```python
from build123d import *

# Parameters (mm, degrees)
SKETCH_1_R      = 23.5
SKETCH_1_R_2    = 8.5
EXTRUDE_1_DEPTH = 15
FILLET_1_R      = 0.8


with BuildPart() as part:
    # 草图1 → 拉伸1 (new body)
    with BuildSketch(Plane(origin=(0, 0, 0), x_dir=(1, 0, 0), z_dir=(0, 1, 0))):
        with Locations(Location((0, 0, 0), (0, 0, 270))):
            Circle(SKETCH_1_R)
        with Locations(Location((0, 0, 0), (0, 0, 270))):
            Circle(SKETCH_1_R_2, mode=Mode.SUBTRACT)
    extrude(amount=EXTRUDE_1_DEPTH)

    # 圆角1
    fillet_1_edges = [part.edges().sort_by_distance(p)[0] for p in [
        (0, 0, -23.5),
        (0, 15, -23.5),
        (0, 0, -8.5),
        (0, 15, -8.5),
    ]]
    fillet(fillet_1_edges, radius=FILLET_1_R)


solid = part.part
```
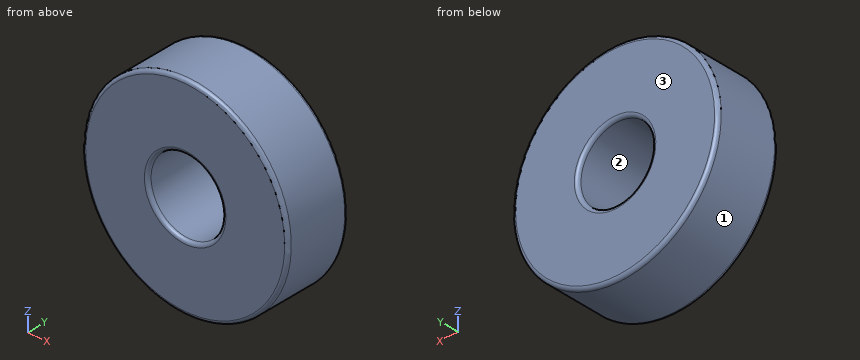
For this review, take the finished solid that the model builds, in its own axes (mm). Face numbers are marked on the shaded views. Round coordinates to 2 decimals unless told otherwise and drop trailing zeros. Write each loop counter-clockwise with the first axis right and the second up, starting at its lowest first coordinate (ties: lowest second). Pieces come first, ordered by that corner, then holes.
1) Insertion check: pin 1 Ø1.5 at (y, z) = (4, -4) entering from -X; pin 2 Ø8 at (y, z) = (9.5, 18.5) entering from +X; pin 3 Ø1 at (x, y) = (-1.5, 7.5) entering from +Z. Each pin has a flat end and moves straight along its axis. Give the tip position at first contact, or say it passes through.
Answer below:
pin 1: stops at x = -23.27
pin 2: stops at x = 18.49
pin 3: stops at z = 23.48
2) Take a section at B-B on x = 0. Give the boundary of the cut face in (y, z).
Answer below:
outline: (0, -22.7) arc R0.8 ccw to (0.8, -23.5) - (14.2, -23.5) arc R0.8 ccw to (15, -22.7) - (15, -9.3) arc R0.8 ccw to (14.2, -8.5) - (0.8, -8.5) arc R0.8 ccw to (0, -9.3) - close; (0, 9.3) arc R0.8 ccw to (0.8, 8.5) - (14.2, 8.5) arc R0.8 ccw to (15, 9.3) - (15, 22.7) arc R0.8 ccw to (14.2, 23.5) - (0.8, 23.5) arc R0.8 ccw to (0, 22.7) - close
3) Mouldability with a two-part tool opening along Z and no side actions: class the marked faces 1, 2 and 3 as +Z half, -Z half, draft (parallel to the pull), parting line (faces both ways), or undercut.
Answer below:
face 1: parting line
face 2: undercut
face 3: draft
4) Take a section at C-C on y = 6.5. Give the boundary of the cut face in (x, z).
Answer below:
outline: circle Ø47 at (0, 0); hole circle Ø17 at (0, 0)
5) For line 1 along X through (y, z) = (5.5, 0); line 2 along Z through (x, y) = (6, 11.25); line 3 along X through (y, z) = (3.75, 7), list the stretches that pass through material, from the lowest coordinate up.
Answer below:
line 1: x = -23.5 to -8.5, 8.5 to 23.5
line 2: z = -22.72 to -6.02, 6.02 to 22.72
line 3: x = -22.43 to -4.82, 4.82 to 22.43
6) Take a section at A-A on z = 0. Give the boundary of the cut face in (x, y).
Answer below:
outline: (-23.5, 0.8) arc R0.8 ccw to (-22.7, 0) - (-9.3, 0) arc R0.8 ccw to (-8.5, 0.8) - (-8.5, 14.2) arc R0.8 ccw to (-9.3, 15) - (-22.7, 15) arc R0.8 ccw to (-23.5, 14.2) - close; (8.5, 0.8) arc R0.8 ccw to (9.3, 0) - (22.7, 0) arc R0.8 ccw to (23.5, 0.8) - (23.5, 14.2) arc R0.8 ccw to (22.7, 15) - (9.3, 15) arc R0.8 ccw to (8.5, 14.2) - close
